Input: part model. Units: mm. Frame: model coordinates. A direction names the side the tool comes from. Coordinates: 2 decimals unless noted, no trailing zeros. Write each loop counter-clockwise with the first axis right and the second up, starting at its lowest first coordinate (ties: lowest second). Pieces come first, ordered by that corner, then holes. Notation, with made-up numbers: (78, 55) -> (132, 55) arc R28 ccw to (132, 91) -> close; hole circle Ø11 at (-29.75, 84). An arc over 180 degrees is marked (long way). Use one line per item in the form item = value. Start each with the question number.
(1) Cut plane A-A on x = -113. Return the cut outline in (y, z).
(2) Ray query, line 1 along Z through (x, y) = (23.5, 3.85); line 2 along X through (y, z) = (1.55, -29); line 3 along X through (y, z) = (7.95, 37). Return the intervals inside material, ascending.
(3) Set-up query: faces 4 (the face through (-110.973, 2.12, 35.141)), 5 (the face through (-108.23, 7.19, 35.5)), 6 (the face through (39, 5, -1)). Return all of +Z, -Z, +X, -X, +Y, -Y with unobstructed straight access to the full face (end or side cutting, diameter ignored); none if empty.
(4) Pull-direction query (X, two-part tool) for faces 1 (the face through (-30, 4, 45)), 2 (the face through (-130, 5, 1)), 3 (the face through (-80.8, 4.3, -34.8)); classes: released by +X, released by -X, zero draft, split by the parting line, or undercut.
(5) First-contact query: pin 1 (3.5 mm diameter, centred on x = -122, z = 0, fed in from +Y); pin 2 (3 mm diameter, centred on x = 110, z = 40.5, fed in from +Y); pin 3 (11.5 mm diameter, centred on x = -113, z = 37, fed in from -Y); pin 4 (9 mm diameter, centred on x = -83, z = 37, fed in from +Y). Flat tips, straight axial feed; report the tip coordinate or a pass-through.
(6) Cut plane B-B on x = 41. Return the cut outline in (y, z), plus the area to 3 significant figures.
```python
from build123d import *

# Parameters (mm, degrees)
SKETCH_1_W                = 260
SKETCH_1_H                = 90
EXTRUDE_1_DEPTH           = 10
CHAMFER_1_SIZE            = 3
HOLE_WIZARD_1_D           = 5.5
HOLE_WIZARD_1_DEPTH       = 10.1
HOLE_WIZARD_1_CBORE_D     = 10
HOLE_WIZARD_1_CBORE_DEPTH = 5.7
HOLE_WIZARD_1_TIP         = 1.652366702
HOLE_WIZARD_M5_1_D        = 4.2
HOLE_WIZARD_M5_1_DEPTH    = 12.4
HOLE_WIZARD_M5_1_TIP      = 1.2618073
SKETCH_8_W                = 180
SKETCH_8_H                = 90
CUT_EXTRUDE_1_DEPTH       = 5
HOLE_WIZARD_M3_1_D        = 2.5
HOLE_WIZARD_M3_1_DEPTH    = 7.5
HOLE_WIZARD_M3_1_TIP      = 0.751075774
HOLE_WIZARD_M4_1_D        = 3.3
HOLE_WIZARD_M4_1_DEPTH    = 20
HOLE_WIZARD_M4_1_TIP      = 0.991420021
HOLE_WIZARD_M4_2_D        = 3.3
HOLE_WIZARD_M4_2_DEPTH    = 20
HOLE_WIZARD_M4_2_TIP      = 0.991420021
MM_1_D                    = 4
MM_1_DEPTH                = 20
MM_1_TIP                  = 1.201721238


with BuildPart() as part:
    # 草图1 → 凸台-拉伸1 (new body)
    with BuildSketch(Plane(origin=(0, 0, 0), x_dir=(1, 0, 0), z_dir=(0, 1, 0))):
        Rectangle(SKETCH_1_W, SKETCH_1_H)
    extrude(amount=EXTRUDE_1_DEPTH)

    # 倒角1
    chamfer_1_edges = [part.edges().sort_by_distance(p)[0] for p in [
        (130, 5, 45),
        (-130, 5, 45),
        (-130, 5, -45),
        (130, 5, -45),
    ]]
    chamfer(chamfer_1_edges, length=CHAMFER_1_SIZE)

    # 打孔尺寸(%根据)内六角圆柱头螺钉的类型1
    with Locations(Plane(origin=(0, 10, 0), x_dir=(1, 0, 0), z_dir=(0, 1, 0))):
        with Locations((-83, 37), (-113, 37), (-83, -37), (-113, -37)):
            CounterBoreHole(HOLE_WIZARD_1_D / 2, HOLE_WIZARD_1_CBORE_D / 2, HOLE_WIZARD_1_CBORE_DEPTH, depth=HOLE_WIZARD_1_DEPTH)
            with Locations((0, 0, -(HOLE_WIZARD_1_DEPTH + HOLE_WIZARD_1_TIP / 2))):  # 118° drill point
                Cone(0, HOLE_WIZARD_1_D / 2, HOLE_WIZARD_1_TIP, mode=Mode.SUBTRACT)

    # M5 螺纹孔1
    with Locations(Plane(origin=(0, 10, 0), x_dir=(1, 0, 0), z_dir=(0, 1, 0))):
        with Locations((-122, 22.5), (-122, 0), (-122, -22.5)):
            Hole(HOLE_WIZARD_M5_1_D / 2, depth=HOLE_WIZARD_M5_1_DEPTH)
            with Locations((0, 0, -(HOLE_WIZARD_M5_1_DEPTH + HOLE_WIZARD_M5_1_TIP / 2))):  # 118° drill point
                Cone(0, HOLE_WIZARD_M5_1_D / 2, HOLE_WIZARD_M5_1_TIP, mode=Mode.SUBTRACT)

    # 草图8 → 切除-拉伸1 (cut)
    with BuildSketch(Plane(origin=(0, 10, 0), x_dir=(1, 0, 0), z_dir=(0, 1, 0))):
        with Locations((40, 0)):
            Rectangle(SKETCH_8_W, SKETCH_8_H)
    extrude(amount=-CUT_EXTRUDE_1_DEPTH, mode=Mode.SUBTRACT)

    # M3 螺纹孔1
    with Locations(Plane(origin=(0, 5, 0), x_dir=(1, 0, 0), z_dir=(0, 1, 0))):
        with Locations((110, -40.5), (90, -40.5), (70, -40.5), (110, 40.5), (90, 40.5), (70, 40.5)):
            Hole(HOLE_WIZARD_M3_1_D / 2, depth=HOLE_WIZARD_M3_1_DEPTH)
            with Locations((0, 0, -(HOLE_WIZARD_M3_1_DEPTH + HOLE_WIZARD_M3_1_TIP / 2))):  # 118° drill point
                Cone(0, HOLE_WIZARD_M3_1_D / 2, HOLE_WIZARD_M3_1_TIP, mode=Mode.SUBTRACT)

    # M4 螺纹孔1
    with Locations(Plane(origin=(0, 5, 0), x_dir=(1, 0, 0), z_dir=(0, 1, 0))):
        with Locations((115, -29), (125, -29), (115, 29), (125, 29)):
            Hole(HOLE_WIZARD_M4_1_D / 2, depth=HOLE_WIZARD_M4_1_DEPTH)
            with Locations((0, 0, -(HOLE_WIZARD_M4_1_DEPTH + HOLE_WIZARD_M4_1_TIP / 2))):  # 118° drill point
                Cone(0, HOLE_WIZARD_M4_1_D / 2, HOLE_WIZARD_M4_1_TIP, mode=Mode.SUBTRACT)

    # M4 螺纹孔2
    with Locations(Plane(origin=(0, 10, 0), x_dir=(1, 0, 0), z_dir=(0, 1, 0))):
        with Locations((30, -25.5), (30, -39.5), (30, 25.5), (30, 39.5)):
            Hole(HOLE_WIZARD_M4_2_D / 2, depth=HOLE_WIZARD_M4_2_DEPTH)
            with Locations((0, 0, -(HOLE_WIZARD_M4_2_DEPTH + HOLE_WIZARD_M4_2_TIP / 2))):  # 118° drill point
                Cone(0, HOLE_WIZARD_M4_2_D / 2, HOLE_WIZARD_M4_2_TIP, mode=Mode.SUBTRACT)

    # 大小mm 暗销孔1
    with Locations(Plane(origin=(0, 5, 0), x_dir=(1, 0, 0), z_dir=(0, 1, 0))):
        with Locations((23.5, -32.5), (36, -32.5), (23.5, 32.5), (36, 32.5)):
            Hole(MM_1_D / 2, depth=MM_1_DEPTH)
            with Locations((0, 0, -(MM_1_DEPTH + MM_1_TIP / 2))):  # 118° drill point
                Cone(0, MM_1_D / 2, MM_1_TIP, mode=Mode.SUBTRACT)


solid = part.part
```
Values:
q1.outline = (0, -45) -> (10, -45) -> (10, -42) -> (4.3, -42) -> (4.3, -39.75) -> (0, -39.75) -> close; (0, -34.25) -> (4.3, -34.25) -> (4.3, -32) -> (10, -32) -> (10, 32) -> (4.3, 32) -> (4.3, 34.25) -> (0, 34.25) -> close; (0, 39.75) -> (4.3, 39.75) -> (4.3, 42) -> (10, 42) -> (10, 45) -> (0, 45) -> close
q2.line_1 = -45 to -34.5, -30.5 to 30.5, 34.5 to 45
q2.line_2 = -130 to 113.35, 116.65 to 123.35, 126.65 to 130
q2.line_3 = -130 to -118, -108 to -88, -78 to -50
q3.face_4 = +Y, -Y
q3.face_5 = +Y
q3.face_6 = +Z, -Z, +X, +Y
q4.face_1 = zero draft
q4.face_2 = released by -X
q4.face_3 = undercut
q5.pin_1 = through
q5.pin_2 = 5
q5.pin_3 = 0
q5.pin_4 = 4.3
q6.outline = (0, -45) -> (5, -45) -> (5, 45) -> (0, 45) -> close
q6.area = 450 mm2
